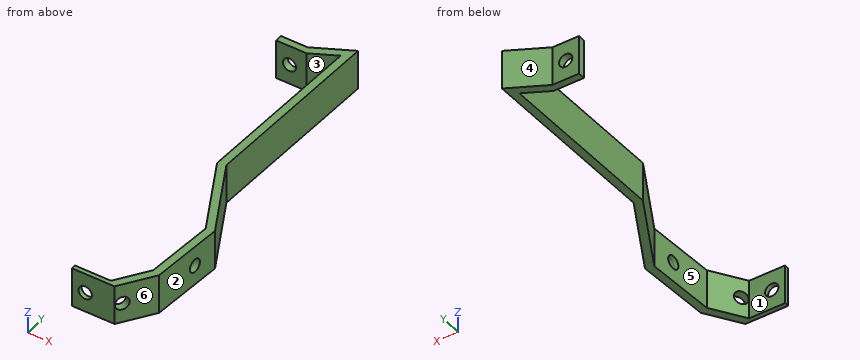
```python
from build123d import *

# Parameters (mm, degrees)
EXTRUDE_1_DEPTH     = 7.5
SKETCH_2_W          = 11.393502177
SKETCH_2_H          = 2.656718216
SKETCH_2_W_2        = 27.04099035
SKETCH_2_H_2        = 1.681293315
EXTRUDE_2_DEPTH     = 15
SKETCH_3_R          = 2.5
CUT_EXTRUDE_1_DEPTH = 5
SKETCH_4_R          = 2.5
CUT_EXTRUDE_2_DEPTH = 10
SKETCH_5_W          = 11
SKETCH_5_H          = 15
CUT_EXTRUDE_3_DEPTH = 3
SKETCH_9_R          = 2.5


with BuildPart() as part:
    # 草图1 → 凸台-拉伸1 (new, symmetric)
    with BuildSketch(Plane.XY):
        Polygon((0, 0), (14, 7.343281784), (12, -62.656718216), (27.393502177, -91.656718216), (25.393502177, -119.656718216), (17.04099035, -132), (14.556387205, -130.318706685), (22.458397846, -118.641172307), (24.339745043, -92.302311555), (8.978589163, -63.363249125), (10.854852, 2.305950198), (1.393502177, -2.656718216), align=None)
    extrude(amount=EXTRUDE_1_DEPTH, both=True)

    # 草图2 → 凸台-拉伸2 (add)
    with BuildSketch(Plane.XY.offset(7.5)):
        with Locations((-4.303248911, -1.328359108)):
            Rectangle(SKETCH_2_W, SKETCH_2_H)
        with Locations((3.520495175, -131.159353342)):
            Rectangle(SKETCH_2_W_2, SKETCH_2_H_2)
    extrude(amount=-EXTRUDE_2_DEPTH)

    # 草图3 → 切除-拉伸1 (cut)
    with BuildSketch(Plane(origin=(0, 0, 0), x_dir=(1, 0, 0), z_dir=(0, 1, 0))):
        with Locations(Location((-5, 0, 0), (0, 0, 270))):
            Circle(SKETCH_3_R)
    extrude(amount=-CUT_EXTRUDE_1_DEPTH, mode=Mode.SUBTRACT)

    # 草图4 → 切除-拉伸2 (cut)
    with BuildSketch(Plane.XZ.offset(132)):
        with Locations(Location((6, 0, 0), (0, 0, 270))):
            Circle(SKETCH_4_R)
    extrude(amount=-CUT_EXTRUDE_2_DEPTH, mode=Mode.SUBTRACT)

    # 草图5 → 切除-拉伸3 (cut)
    with BuildSketch(Plane.XZ.offset(132)):
        with Locations((-4.5, 0)):
            Rectangle(SKETCH_5_W, SKETCH_5_H)
    extrude(amount=-CUT_EXTRUDE_3_DEPTH, mode=Mode.SUBTRACT)

    # 草图9 → 切除-旋转1 (revolve, cut)
    with BuildSketch(Plane(origin=(33.768124273, -2.412008877, 0), x_dir=(0, 0, -1), z_dir=(0.997458699830735, -0.07124704998790972, 0)), mode=Mode.PRIVATE) as cut_revolve_1_sk:
        with Locations((0, -99.543422459)):
            Circle(SKETCH_9_R)
    revolve(cut_revolve_1_sk.sketch.rotate(Axis((25.607243327, -116.664342117, 0), (0, 0, 1)), 6.860802101), axis=Axis((25.607243327, -116.664342117, 0), (0, 0, 1)), mode=Mode.SUBTRACT)


solid = part.part
```
Could you check a few things on this model? Use its own coordinates, in mm. Face numbers are marked on the shaded views. A direction names the side the tool comes from. Give positions to 0.01 mm unless a question says otherwise; leave off trailing zeros. Loops run counter-clockwise (first coordinate to the right, second up) from the corner with the lowest first, then second, coordinate; pieces in that order, holes last. Notation, with made-up numbers: (6.5, -3.75) -> (57.5, -3.75) arc R29 cw to (57.5, 34.25) -> close; hole circle Ø3 at (47, 76). An arc over 180 degrees is marked (long way). Put each result on its own line as item: value.
(1) I'm going to push flat-ended pins straight in: pin 1 Ø1 at (y, z) = (-89.5, 5) entering from -X; pin 2 Ø8 at (x, z) = (-5, 0) entering from -Y; pin 3 Ø3.5 at (x, z) = (-5.5, 0.5) entering from -Y; pin 4 Ø5 at (x, z) = (21, 0) entering from +Y. Where does each tip first touch, or does it pass through?
Computed:
pin 1: x = 22.59
pin 2: y = -2.66
pin 3: through
pin 4: y = -74.9
(2) Please list where these lines run through material, in increasing order: probe 1 along X at (y, z) = (-1.6, 0); probe 2 along X at (y, z) = (-0.6, 0); probe 3 along Y at (x, z) = (-8, -4.5). Write a range as [from, to].
Computed:
probe 1: [-10, -7.5], [-2.5, 3.41], [10.74, 13.74]
probe 2: [-10, -7.5], [-2.5, 5.31], [10.77, 13.77]
probe 3: [-2.66, 0]
(3) Imagine slicing it at C-C on z = 0. State how many separate pieces and enclosed holes the cut face has, plus the area to 3 significant figures.
Computed:
separate pieces: 5
enclosed holes: 0
area: 468 mm^2
(4) Thinking about a two-plate mould opening in Y: for the marked faces 3, 4, 5 and 6, which applies, pulls with the +Y half, pulls with the -Y half, needs draft (parallel to the pull), parting line crosses it, or undercut?
Computed:
face 3: undercut
face 4: pulls with the +Y half
face 5: undercut
face 6: pulls with the -Y half
(5) Imagine slicing it at D-D on y = -73.5. Write out the boundary of the cut face in (x, z).
Computed:
outline: (14.36, -7.5) -> (17.76, -7.5) -> (17.76, 7.5) -> (14.36, 7.5) -> close
(6) Imagine slicing it at B-B on z = 5.5. Write out the boundary of the cut face in (x, y).
Computed:
outline: (-10, -2.66) -> (1.39, -2.66) -> (10.85, 2.31) -> (8.98, -63.36) -> (24.34, -92.3) -> (22.46, -118.64) -> (14.56, -130.32) -> (1, -130.32) -> (1, -132) -> (17.04, -132) -> (25.39, -119.66) -> (27.39, -91.66) -> (12, -62.66) -> (14, 7.34) -> (0, 0) -> (-10, 0) -> close
(7) For the marked faces 1 and 2, which set-ups out of +Z, -Z, +X, -X, +Y, -Y let a thin tool reach every point of the face, with its end or its side?
Computed:
face 1: +Z, -Z, -X
face 2: +Z, -Z, +X, -Y
(8) Imagine slicing it at A-A on x = -5. Write out the boundary of the cut face in (y, z), plus the area to 3 significant figures.
Computed:
outline: (-2.66, -7.5) -> (0, -7.5) -> (0, -2.5) -> (-2.66, -2.5) -> close; (-2.66, 2.5) -> (0, 2.5) -> (0, 7.5) -> (-2.66, 7.5) -> close
area: 26.6 mm^2
